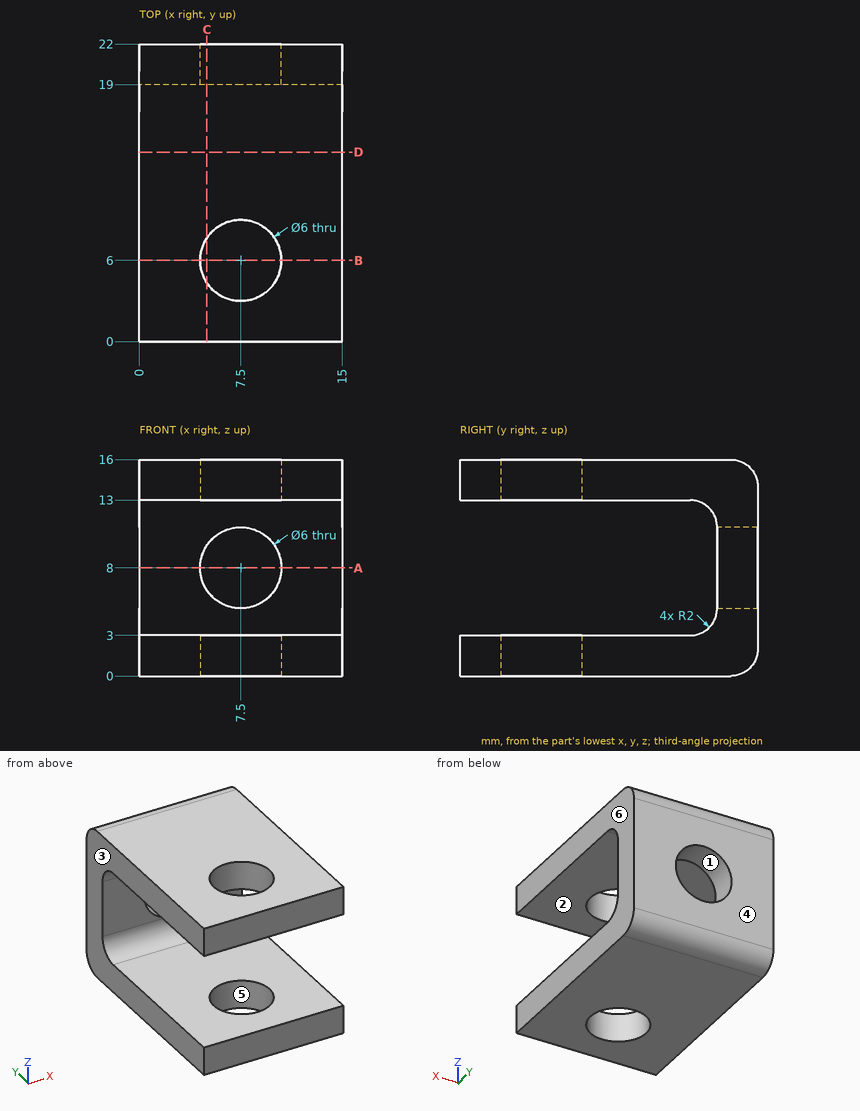
Could you check a few things on this drawing? It's one solid part, dimensions in mm from its lowest x, y, z. A direction names the side the tool comes from. Round coordinates to 2 decimals unless told otherwise and drop trailing zeros. Loops run counter-clockwise (first coordinate to the right, second up) from the corner with the lowest first, then second, coordinate; pieces in that order, holes last. Notation, with made-up numbers: M 6.25,71 L 33.25,71 A28 ccw 33.25,102 Z; hole C 78,70.25 d10. An arc over 180 degrees is marked long. Write item = value, one per line. Start each with the question number.
(1) Suppose I cut it at A-A on z = 8. Write out the boundary of the cut face in (x, y).
(2) I need wall thicknesses on line 1 along Z through (x, y) = (7, 15); line 2 along X through (y, z) = (21.1, 8); line 3 along Y through (x, z) = (11.75, 10.25). Which ranges of each line are inside material? Lowest first, please.
(3) Suppose I cut it at B-B on y = 6. Write out the boundary of the cut face in (x, z), plus the area to 3 significant figures.
(4) Suppose I cut it at C-C on x = 5. Write out the boundary of the cut face in (y, z), plus the area to 3 significant figures.
(5) Suppose I cut it at D-D on y = 14. Write out the boundary of the cut face in (x, z).
(6) If we mould it in two halves opening along X, with no side actions, what happens to the marked faces 3, 4, 5 and 6? For each: released by +X, released by -X, zero draft, split by the parting line, or undercut.
(7) I'm going to push flat-ended pins straight in: P1, Ø1.8, axis at x = 12, z = 8, coming from the -Y side; P2, Ø3, axis at x = 5.5, z = 5, coming from the -Y side. Where does each tip first touch, or does it pass through?
(8) Which directions (+Z, -Z, +X, -X, +Y, -Y) give clear straight access to the entire face, cutting with the end or side of a thin tool? Please do the marked faces 1 and 2.
Answer block:
q1.outline = M 0,19 L 4.5,19 L 4.5,22 L 0,22 Z; M 10.5,19 L 15,19 L 15,22 L 10.5,22 Z
q2.line_1 = 0 to 3, 13 to 16
q2.line_2 = 0 to 4.5, 10.5 to 15
q2.line_3 = 19 to 22
q3.outline = M 0,0 L 4.5,0 L 4.5,3 L 0,3 Z; M 0,13 L 4.5,13 L 4.5,16 L 0,16 Z; M 10.5,0 L 15,0 L 15,3 L 10.5,3 Z; M 10.5,13 L 15,13 L 15,16 L 10.5,16 Z
q3.area = 54.0 mm²
q4.outline = M 0,0 L 4.34,0 L 4.34,3 L 0,3 Z; M 0,13 L 4.34,13 L 4.34,16 L 0,16 Z; M 7.66,0 L 20,0 A2 ccw 22,2 L 22,6.34 L 19,6.34 L 19,5 A2 cw 17,3 L 7.66,3 Z; M 7.66,13 L 17,13 A2 cw 19,11 L 19,9.66 L 22,9.66 L 22,14 A2 ccw 20,16 L 7.66,16 Z
q4.area = 132 mm²
q5.outline = M 0,0 L 15,0 L 15,3 L 0,3 Z; M 0,13 L 15,13 L 15,16 L 0,16 Z
q6.face_3 = released by -X
q6.face_4 = zero draft
q6.face_5 = undercut
q6.face_6 = released by +X
q7.P1 = 19
q7.P2 = 18.32
q8.face_1 = +Y, -Y
q8.face_2 = +X, -X, -Y
